```python
from build123d import *


with BuildPart() as part:
    # 草图1 → 旋转1 (revolve)
    with BuildSketch(Plane.XY, mode=Mode.PRIVATE) as revolve_1_sk:
        Polygon((0, 0), (0, 17.5), (50, 17.5), (50, 20), (85, 20), (85, 60), (935, 60), (935, 20), (970, 20), (970, 17.5), (1027, 17.5), (1027, 0), align=None)
    revolve(revolve_1_sk.sketch.rotate(Axis((1027, 0, 0), (-1, 0, 0)), 90), axis=Axis((1027, 0, 0), (-1, 0, 0)))


solid = part.part
```
The model under review builds one solid part; all positions refer to its coordinate system, in mm. A direction names the side the tool comes from. Round coordinates to 2 decimals unless told otherwise and drop trailing zeros. Loops run counter-clockwise (first coordinate to the right, second up) from the corner with the lowest first, then second, coordinate; pieces in that order, holes last. Notation, with made-up numbers: (1, 7.25) -> (29, 7.25) arc R16 cw to (29, 38.25) -> close; hole circle Ø5 at (-12.5, 36). An arc over 180 degrees is marked (long way). Answer as a JSON object with one key per item and string values. Group by question number.
1) We need section A-A on y = 0. Write out the cut boundary in (x, z), then the cut area to 3 significant figures.
2) For faces 1 (the face through (1027, 0, 0)), 2 (the face through (67.74, -0.88, 19.98)), 3 (the face through (970, 18, 0)), list the 3-axis set-ups (+Z, -Z, +X, -X, +Y, -Y) from which the entire face can be reached by the end or side of a thin tool; tool diameter is ignored.
3) For pin 1 Ø5 at (y, z) = (-8, -45.5) entering from -X; pin 2 Ø6 at (x, z) = (514, -35.5) entering from +Y; pin 3 Ø2 at (x, y) = (578, -4.5) entering from +Z, all flat-tipped, find the tip position at first contact; note any pin that passes through.
4) We need section C-C on x = 313.5. Write out the cut boundary in (y, z).
5) We need section D-D on z = -48. Write out the cut boundary in (x, y).
6) For line 1 (X direction, y = -21, z = 50.5); line 2 (Z direction, x = 314.5, y = 0.5); line 3 (Y direction, x = 266, z = -24), list the stretches that pass through material, from the lowest coordinate up. Write a range as [from, to].
Result set:
{
 "1": {"outline": "(0, -17.5) -> (50, -17.5) -> (50, -20) -> (85, -20) -> (85, -60) -> (935, -60) -> (935, -20) -> (970, -20) -> (970, -17.5) -> (1027, -17.5) -> (1027, 17.5) -> (970, 17.5) -> (970, 20) -> (935, 20) -> (935, 60) -> (85, 60) -> (85, 20) -> (50, 20) -> (50, 17.5) -> (0, 17.5) -> close", "area": "109,000 mm²"},
 "2": {"face 1": "+Z, -Z, +X, +Y, -Y", "face 2": "-X", "face 3": "+X"},
 "3": {"pin 1": "x = 85", "pin 2": "y = 50.44", "pin 3": "z = 59.9"},
 "4": {"outline": "circle Ø120 at (0, 0)"},
 "5": {"outline": "(85, -36) -> (935, -36) -> (935, 36) -> (85, 36) -> close"},
 "6": {"line 1": "[85, 935]", "line 2": "[-60, 60]", "line 3": "[-54.99, 54.99]"}
}
